Read the model definition and answer for the solid it produces. Units are mm, in the model's axes. A direction names the side the tool comes from. Give positions to 0.01 mm unless a question says otherwise; leave off trailing zeros. Write each loop counter-clockwise with the first axis right and the second up, starting at its lowest first coordinate (ties: lowest second). Pieces come first, ordered by that corner, then holes. Notation, with made-up numbers: (37.25, 80.25) -> (92.25, 80.25) arc R24 cw to (92.25, 104.25) -> close; hole circle Ø2 at (-38, 16). An arc over 180 degrees is marked (long way). Answer as CSV lines item,"result". Start each with the question number.
1. For a pull along X with two mould halves and no side action, classify faces 3 (the flat face through (374, 507, 456.3)), 4 (the flat face through (209.166, 507, 264)), 5 (the flat face through (306.414, 507.395, 339.786)) as pulls with the +X half, pulls with the -X half, needs draft (parallel to the pull), parting line crosses it, or undercut.
2. Given pin 1 (4.5 mm diameter, centred on y = 507.5, z = 446, fed in from -X); pin 2 (2 mm diameter, centred on y = 508, z = 290.5, fed in from +X); pin 3 (4 mm diameter, centred on y = 502, z = 311.5, fed in from +X), each flat-ended and moving along its own axis, determine where each tip first touches the part or whether it passes through.
3. The part is cut by section A-A, the plane y = 503. Determine the outline of the cut face in (x, z), and give its area (3 significant figures).
4. A tool of negligible diameter and unlimited length cuts with its end or side. For faces 1 (the flat face through (306, 500, 345)), 2 (the flat face through (371.666, 507, 439)), from which of +Z, -Z, +X, -X, +Y, -Y can it reach the whole face along a straight path? Write none if from no direction.
5. Find the intervals of material crossed by line 1 (Z direction, x = 225, y = 502); line 2 (Z direction, x = 328.5, y = 504.75); line 3 (X direction, y = 507.75, z = 333.5), in increasing order.
6. The part is cut by section C-C, the plane x = 224. Determine the outline of the cut face in (y, z).
7. The part is cut by section B-B, the plane z = 436.5. Determine the outline of the cut face in (x, y), and give its area (3 significant figures).
from build123d import *

# Parameters (mm, degrees)
BOSS_EXTRUDE1_DEPTH = 15


with BuildPart() as part:
    # Sketch1 → Boss-Extrude1 (new body)
    with BuildSketch(Plane.XZ.offset(-500)):
        Polygon((376.666458359, 456.299687539), (376.666458359, 416.299687539), (234.166458359, 261.099687539), (209.166458359, 261.099687539), (209.166458359, 266.099687539), (227.89663092, 266.099687539), (361.870871539, 412.014088551), (371.666458359, 422.682685565), (371.666458359, 456.299687539), align=None)
    extrude(amount=-BOSS_EXTRUDE1_DEPTH)


solid = part.part
Results found:
1,face 3,"needs draft"
1,face 4,"pulls with the -X half"
1,face 5,"pulls with the +X half"
2,pin 1,"stops at x = 371.67"
2,pin 2,"stops at x = 262.08"
2,pin 3,"stops at x = 282.28"
3,outline,"(209.17, 261.1) -> (234.17, 261.1) -> (376.67, 416.3) -> (376.67, 456.3) -> (371.67, 456.3) -> (371.67, 422.68) -> (227.9, 266.1) -> (209.17, 266.1) -> close"
3,area,"1,990 mm²"
4,face 1,"+Z, -Z, +X, -X, -Y"
4,face 2,"+Z, -X, +Y, -Y"
5,line 1,"z = 261.1 to 266.1"
5,line 2,"z = 363.84 to 375.67"
5,line 3,"x = 289.78 to 300.64"
6,outline,"(500, 261.1) -> (515, 261.1) -> (515, 266.1) -> (500, 266.1) -> close"
7,outline,"(371.67, 500) -> (376.67, 500) -> (376.67, 515) -> (371.67, 515) -> close"
7,area,"75.0 mm²"
